from build123d import *

# Parameters (mm, degrees)
BOSS_EXTRUDE1_DEPTH   = 50
M8X1_0_TAPPED_HOLE1_D = 7
CUT_EXTRUDE1_DEPTH    = 57.010506805
CUT_EXTRUDE2_DEPTH    = 4
FILLET1_R             = 3


with BuildPart() as part:
    # Sketch1 → Boss-Extrude1 (new body)
    with BuildSketch(Plane(origin=(0, 0, 0), x_dir=(1, 0, 0), z_dir=(0, 1, 0))):
        with BuildLine():
            Line((-22.5, 84.557672626), (-22.5, 96))
            Line((-22.5, 96), (22.5, 96))
            Line((22.5, 96), (22.5, 84.557672626))
            ThreePointArc((22.5, 84.557672626), (0, 87.5), (-22.5, 84.557672626))
        make_face()
    extrude(amount=BOSS_EXTRUDE1_DEPTH)

    # M8x1.0 Tapped Hole1 (through all)
    with Locations(Plane(origin=(0, 0, -96), x_dir=(-1, 0, 0), z_dir=(0, 0, -1))):
        with Locations((-14.5, 25), (14.5, 25)):
            Hole(M8X1_0_TAPPED_HOLE1_D / 2)

    # Sketch4 → Cut-Extrude1 (cut, through all)
    with BuildSketch(Plane(origin=(0, 0, -96), x_dir=(-1, 0, 0), z_dir=(0, 0, -1))):
        with BuildLine():
            Line((2.25, 45), (2.25, 5))
            ThreePointArc((2.25, 5), (0, 2.75), (-2.25, 5))
            Line((-2.25, 5), (-2.25, 45))
            ThreePointArc((-2.25, 45), (0, 47.25), (2.25, 45))
        make_face()
    extrude(amount=-CUT_EXTRUDE1_DEPTH, mode=Mode.SUBTRACT)

    # Sketch5 → Cut-Extrude2 (cut)
    with BuildSketch(Plane(origin=(0, 0, -96), x_dir=(-1, 0, 0), z_dir=(0, 0, -1))):
        with BuildLine():
            Line((4, 45), (4, 5))
            ThreePointArc((4, 5), (0, 1), (-4, 5))
            Line((-4, 5), (-4, 45))
            ThreePointArc((-4, 45), (0, 49), (4, 45))
        make_face()
    extrude(amount=-CUT_EXTRUDE2_DEPTH, mode=Mode.SUBTRACT)

    # Fillet1
    fillet1_edges = [part.edges().sort_by_distance(p)[0] for p in [
        (22.5, 50, -90.278836313),
        (22.5, 0, -90.278836313),
        (-22.5, 0, -90.278836313),
        (-22.5, 50, -90.278836313),
    ]]
    fillet(fillet1_edges, radius=FILLET1_R)


solid = part.part
Verification items for the finished model (mm, model axes). A direction names the side the tool comes from. Give positions to 0.01 mm unless a question says otherwise; leave off trailing zeros. Write each loop counter-clockwise with the first axis right and the second up, starting at its lowest first coordinate (ties: lowest second). Pieces come first, ordered by that corner, then holes. Notation, with made-up numbers: (-27, 41.5) -> (15, 41.5) arc R17 cw to (15, 55.5) -> close; hole circle Ø6 at (52.5, 41.5). An arc over 180 degrees is marked (long way). Use CSV: the item, a comma, the result in double quotes.
(1) Sectioned sample at A-A (y = 19). Record the cut outline in (x, z).
Derived:
outline,"(-22.5, -96) -> (-4, -96) -> (-4, -92) -> (-2.25, -92) -> (-2.25, -87.47) arc R87.5 cw to (-22.5, -84.56) -> close; (2.25, -92) -> (4, -92) -> (4, -96) -> (22.5, -96) -> (22.5, -84.56) arc R87.5 cw to (2.25, -87.47) -> close"
(2) Material ranges on L1, parallel to X at y = 25, z = -89.5; L2, parallel to X at y = 25, z = -93; L3, parallel to X at y = 9.5, z = -90.5, recorded low to high.
Derived:
L1,"x = -22.5 to -18, -11 to -2.25, 2.25 to 11, 18 to 22.5"
L2,"x = -22.5 to -18, -11 to -4, 4 to 11, 18 to 22.5"
L3,"x = -22.5 to -2.25, 2.25 to 22.5"
(3) Release check for a two-part mould opening along X. For faces 4 (the cylindrical face through (-0.05, 2.75, -89.77)), 5 (the cylindrical face through (21.6, 0.86, -90.2)), 6 (the flat face through (5, 25, -96)) record: +X half, -X half, draft (parallel to the pull), parting line (faces both ways), or undercut.
Derived:
face 4,"undercut"
face 5,"+X half"
face 6,"draft"
(4) Set-up check for faces 1 (the flat face through (2.25, 25, -90)), 2 (the flat face through (-3, 25, -92)), 3 (the cylindrical face through (21.6, 49.14, -90.2)): record each of +Z, -Z, +X, -X, +Y, -Y from which the full face is reachable in a straight line by a thin tool's end or side.
Derived:
face 1,"+Z, -Z"
face 2,"-Z"
face 3,"+Z, -Z, +X, +Y"
(5) Sectioned sample at D-D (y = 25). Record the cut outline in (x, z), plus the area to 3 significant figures.
Derived:
outline,"(-22.5, -96) -> (-18, -96) -> (-18, -85.63) arc R87.5 cw to (-22.5, -84.56) -> close; (-11, -96) -> (-4, -96) -> (-4, -92) -> (-2.25, -92) -> (-2.25, -87.47) arc R87.5 cw to (-11, -86.81) -> close; (2.25, -92) -> (4, -92) -> (4, -96) -> (11, -96) -> (11, -86.81) arc R87.5 cw to (2.25, -87.47) -> close; (18, -96) -> (22.5, -96) -> (22.5, -84.56) arc R87.5 cw to (18, -85.63) -> close"
area,"238 mm^2"
(6) Sectioned sample at B-B (x = 0). Record the cut outline in (y, z), plus the area to 4 significant figures.
Derived:
outline,"(0, -96) -> (1, -96) -> (1, -92) -> (2.75, -92) -> (2.75, -87.5) -> (0, -87.5) -> close; (47.25, -92) -> (49, -92) -> (49, -96) -> (50, -96) -> (50, -87.5) -> (47.25, -87.5) -> close"
area,"32.75 mm^2"
(7) Go/stop test with flat-tipped pins: pin 1 (2.5 mm diameter, centred on x = -1.5, y = 35, fed in from -Z); pin 2 (5 mm diameter, centred on x = -14.5, y = 6, fed in from +Z). Record where each tip stops, or that it passes through.
Derived:
pin 1,"stops at z = -92"
pin 2,"stops at z = -85.83"
(8) Sectioned sample at C-C (z = -94.5). Record the cut outline in (x, y), plus the area to 3 significant figures.
Derived:
outline,"(-22.5, 3) arc R3 ccw to (-19.5, 0) -> (19.5, 0) arc R3 ccw to (22.5, 3) -> (22.5, 47) arc R3 ccw to (19.5, 50) -> (-19.5, 50) arc R3 ccw to (-22.5, 47) -> close; hole circle Ø7 at (-14.5, 25); hole (-4, 5) arc R4 ccw to (4, 5) -> (4, 45) arc R4 ccw to (-4, 45) -> close; hole circle Ø7 at (14.5, 25)"
area,"1,800 mm^2"
